Could you check a few things on this model? Use its own coordinates, in mm. Round coordinates to 2 decimals unless told otherwise and drop trailing zeros. Loops run counter-clockwise (first coordinate to the right, second up) from the corner with the lowest first, then second, coordinate; pieces in that order, holes last. Notation, with made-up numbers: (-4.5, -7) -> (27.5, -7) arc R23 ccw to (27.5, 12) -> close; hole circle Ø6 at (41.5, 58). An arc over 180 degrees is marked (long way). One line per item, written item: value.
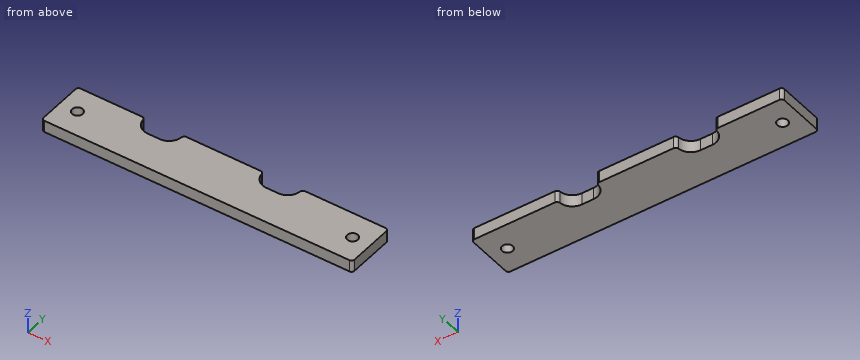
```python
from build123d import *

# Parameters (mm, degrees)
SKETCH1_R           = 9
BOSS_EXTRUDE1_DEPTH = 20


with BuildPart() as part:
    # Sketch1 → Boss-Extrude1 (new body)
    with BuildSketch(Plane.XY):
        with BuildLine():
            Line((-26685.045416981, 9467.963220498), (-26685.045416981, 9542.963223042))
            ThreePointArc((-26685.045416981, 9542.963223042), (-26683.580949969, 9546.498755277), (-26680.045416963, 9547.96322043))
            Line((-26680.045416963, 9547.96322043), (-26576.431543676, 9547.96322043))
            ThreePointArc((-26576.431543676, 9547.96322043), (-26573.060544526, 9546.655965332), (-26571.452248862, 9543.417765798))
            ThreePointArc((-26571.452248862, 9543.417765798), (-26564.214913831, 9528.845869116), (-26549.045416948, 9522.963220428))
            Line((-26549.045416948, 9522.963220428), (-26529.045416963, 9522.963220428))
            ThreePointArc((-26529.045416963, 9522.963220428), (-26513.875918272, 9528.845870766), (-26506.638584632, 9543.417770687))
            ThreePointArc((-26506.638584632, 9543.417770687), (-26505.030289423, 9546.655967321), (-26501.659292496, 9547.963220408))
            Line((-26501.659292496, 9547.963220408), (-26376.431544058, 9547.963220408))
            ThreePointArc((-26376.431544058, 9547.963220408), (-26373.060544852, 9546.655965256), (-26371.452248862, 9543.417765804))
            ThreePointArc((-26371.452248862, 9543.417765804), (-26364.214913847, 9528.845869098), (-26349.045416954, 9522.963220397))
            Line((-26349.045416954, 9522.963220397), (-26329.045416961, 9522.963220397))
            ThreePointArc((-26329.045416961, 9522.963220397), (-26313.875920919, 9528.845868323), (-26306.638585232, 9543.417763496))
            ThreePointArc((-26306.638585232, 9543.417763496), (-26305.03028784, 9546.655964088), (-26301.659287339, 9547.963220451))
            Line((-26301.659287339, 9547.963220451), (-26289.045416951, 9547.963220451))
            Line((-26289.045416951, 9547.963220451), (-26166.045416928, 9547.963220451))
            ThreePointArc((-26166.045416928, 9547.963220451), (-26162.509883026, 9546.498754363), (-26161.045416939, 9542.96322046))
            Line((-26161.045416939, 9542.96322046), (-26161.045416939, 9467.96322112))
            ThreePointArc((-26161.045416939, 9467.96322112), (-26162.509882821, 9464.42768677), (-26166.045416981, 9462.96322043))
            Line((-26166.045416981, 9462.96322043), (-26680.045417049, 9462.96322043))
            ThreePointArc((-26680.045417049, 9462.96322043), (-26683.580950913, 9464.427686595), (-26685.045416981, 9467.963220498))
        make_face()
        with Locations((-26655.045416981, 9505.46322043)):
            Circle(SKETCH1_R, mode=Mode.SUBTRACT)
        with Locations((-26191.045416981, 9505.46322043)):
            Circle(SKETCH1_R, mode=Mode.SUBTRACT)
    extrude(amount=BOSS_EXTRUDE1_DEPTH)


solid = part.part
```
Item 1: Will these pins go through, and if not, where does the flat tip stop? pin 1 Ø10 at (x, z) = (-26539, 9.5) entering from +Y; pin 2 Ø14.5 at (x, y) = (-26655.05, 9505.46) entering from -Z.
Output:
pin 1: stops at y = 9522.96
pin 2: passes through
Item 2: If we section it at A-A on y = 9537: List the corners of the cut face in (x, z) for me, plus the area to 3 significant figures.
Output:
outline: (-26685.05, 0) -> (-26569.89, 0) -> (-26569.89, 20) -> (-26685.05, 20) -> close; (-26508.2, 0) -> (-26369.89, 0) -> (-26369.89, 20) -> (-26508.2, 20) -> close; (-26308.2, 0) -> (-26161.05, 0) -> (-26161.05, 20) -> (-26308.2, 20) -> close
area: 8,010 mm²
Item 3: If we section it at B-B on z = 14.75: List the corners of the cut face in (x, y) for me, plus the area to 3 significant figures.
Output:
outline: (-26685.05, 9467.96) arc R5 ccw to (-26680.05, 9462.96) -> (-26166.05, 9462.96) arc R5 ccw to (-26161.05, 9467.96) -> (-26161.05, 9542.96) arc R5 ccw to (-26166.05, 9547.96) -> (-26301.66, 9547.96) arc R5 ccw to (-26306.64, 9543.42) arc R22.5 cw to (-26329.05, 9522.96) -> (-26349.05, 9522.96) arc R22.5 cw to (-26371.45, 9543.42) arc R5 ccw to (-26376.43, 9547.96) -> (-26501.66, 9547.96) arc R5 ccw to (-26506.64, 9543.42) arc R22.5 cw to (-26529.05, 9522.96) -> (-26549.05, 9522.96) arc R22.5 cw to (-26571.45, 9543.42) arc R5 ccw to (-26576.43, 9547.96) -> (-26680.05, 9547.96) arc R5 ccw to (-26685.05, 9542.96) -> close; hole circle Ø18 at (-26655.05, 9505.46); hole circle Ø18 at (-26191.05, 9505.46)
area: 41,200 mm²
Item 4: If we section it at C-C on x = -26524: List the corners of the cut face in (y, z) for me, plus the area to 3 significant figures.
Output:
outline: (9462.96, 0) -> (9523.54, 0) -> (9523.54, 20) -> (9462.96, 20) -> close
area: 1,210 mm²
Item 5: I need wall thicknesses on line 1 (X direction, y = 9505.5, z = 11); line 2 (X direction, y = 9535, z = 5.5); line 3 (Y direction, x = -26560, z = 7.75). Which ranges of each line are inside material? Lowest first, please. Write a range as from..to.
Output:
line 1: x = -26685.05..-26664.05, -26646.05..-26200.05, -26182.05..-26161.05
line 2: x = -26685.05..-26568.96, -26509.13..-26368.96, -26309.13..-26161.05
line 3: y = 9462.96..9525.81
